```python
from build123d import *

# Parameters (mm, degrees)
BOSS_EXTRUDE1_DEPTH = 101.6
BOSS_EXTRUDE2_START = 50.8
BOSS_EXTRUDE2_DEPTH = 50.8
CUT_EXTRUDE1_DEPTH  = 800


with BuildPart() as part:
    # Sketch1 → Boss-Extrude1 (new body)
    with BuildSketch(Plane.XY):
        with BuildLine():
            Line((0, 254), (1473.2, 254))
            ThreePointArc((1473.2, 254), (1580.963073453, 209.363073453), (1625.6, 101.6))
            Line((1625.6, 101.6), (1625.6, -254))
            Line((1625.6, -254), (1623.6, -254))
            Line((1623.6, -254), (1623.6, 101.6))
            ThreePointArc((1623.6, 101.6), (1579.54885989, 207.94885989), (1473.2, 252))
            Line((1473.2, 252), (0, 252))
            ThreePointArc((0, 252), (-178.190908859, 178.190908859), (-252, 0))
            Line((-252, 0), (-254, 0))
            ThreePointArc((-254, 0), (-179.605122421, 179.605122421), (0, 254))
        make_face()
    extrude(amount=-BOSS_EXTRUDE1_DEPTH)

    # Sketch2 → Boss-Extrude2 (add)
    with BuildSketch(Plane.XY.offset(BOSS_EXTRUDE2_START)):
        with BuildLine():
            Line((1625.6, -254), (1625.6, 101.6))
            ThreePointArc((1625.6, 101.6), (1580.963073453, 209.363073453), (1473.2, 254))
            Line((1473.2, 254), (1320.8, 254))
            ThreePointArc((1320.8, 254), (1213.036926547, 209.363073453), (1168.4, 101.6))
            Line((1168.4, 101.6), (1168.4, -254))
            Line((1168.4, -254), (1170.4, -254))
            Line((1170.4, -254), (1170.4, 101.6))
            ThreePointArc((1170.4, 101.6), (1214.45114011, 207.94885989), (1320.8, 252))
            Line((1320.8, 252), (1473.2, 252))
            ThreePointArc((1473.2, 252), (1579.54885989, 207.94885989), (1623.6, 101.6))
            Line((1623.6, 101.6), (1623.6, -254))
            Line((1623.6, -254), (1625.6, -254))
        make_face()
    extrude(amount=-BOSS_EXTRUDE2_DEPTH)

    # Sketch3 → Cut-Extrude1 (cut)
    with BuildSketch(Plane(origin=(0, 0, 0), x_dir=(0, 0, -1), z_dir=(1, 0, 0))):
        with BuildLine():
            Line((101.6, 172.72), (101.6, 0))
            Line((101.6, 0), (0, 0))
            ThreePointArc((0, 0), (44.901280605, 18.598719395), (63.5, 63.5))
            Line((63.5, 63.5), (63.5, 134.62))
            ThreePointArc((63.5, 134.62), (74.659231637, 161.560768363), (101.6, 172.72))
        make_face()
    extrude(amount=-CUT_EXTRUDE1_DEPTH, mode=Mode.SUBTRACT)


solid = part.part
```
Design review of the part built by this model. Coordinates are the model's own, in mm. A direction names the side the tool comes from. Round coordinates to 2 decimals unless told otherwise and drop trailing zeros. Write each loop counter-clockwise with the first axis right and the second up, starting at its lowest first coordinate (ties: lowest second). Pieces come first, ordered by that corner, then holes. Notation, with made-up numbers: (85, 23.25) -> (140, 23.25) arc R31 cw to (140, 56.25) -> close; hole circle Ø5 at (19.5, 32). An arc over 180 degrees is marked (long way). Write item = value, one per line. Start each with the question number.
1) Take a section at C-C, the plane x = 1395. State the section outline as (y, z) points.
2) Take a section at B-B, the plane z = -41.5. State the section outline as (x, y) points.
3) Wall thickness on probe 1 along X at (y, z) = (58, 10); probe 2 along X at (y, z) = (-173, -31); probe 3 along Y at (x, z) = (896, -48): over which ranges is each line inside the solid? List them lowest first. Write a range as from..to.
4) Tool access review of faces 5 (the face through (-232, 99, -63.5)), 6 (the face through (1168.4, -74, 26)), 7 (the face through (1578.373, 209.112, -24.333)), 8 (the face through (-251.9, 18.4, -44.7)), 9 (the face through (1582.141, 208.172, -24.333)): name each direction out of +Z, -Z, +X, -X, +Y, -Y from which nothing blocks a thin tool from reaching the whole face with its end or side.
5) Take a section at A-A, the plane y = 197.5. State the section outline as (x, z) points.
6) Take a section at D-D, the plane y = 31.5. State the section outline as (x, z) points.
7) Mouldability with a two-part tool opening along X and no side actions: class faces 1 (the face through (1623.6, -74, -24)), 2 (the face through (-147.97, 206.45, -38.8)), 3 (the face through (1625.6, -79, -24)), 4 (the face through (747, 254, -41)) as +X half, -X half, draft (parallel to the pull), parting line (faces both ways), or undercut.
8) Clearance check with flat-ended pins moving along their axes: pin 1 (3 mm diameter, centred on x = 663, z = -18.5, fed in from -Y); pin 2 (2 mm diameter, centred on y = 187, z = -19, fed in from -X); pin 3 (16.5 mm diameter, centred on x = -231.5, y = 88.5, fed in from -Z). State where each tip first meets the part, or that it passes through.
Results list:
q1.outline = (252, -101.6) -> (254, -101.6) -> (254, 50.8) -> (252, 50.8) -> close
q2.outline = (-253.53, 15.44) -> (-251.53, 15.44) arc R252 cw to (0, 252) -> (1473.2, 252) arc R150.4 cw to (1623.6, 101.6) -> (1623.6, -254) -> (1625.6, -254) -> (1625.6, 101.6) arc R152.4 ccw to (1473.2, 254) -> (0, 254) arc R254 ccw to start
q3.probe_1 = 1168.4..1170.4, 1623.6..1625.6
q3.probe_2 = 1623.6..1625.6
q3.probe_3 = 252..254
q4.face_5 = -Z, -X, +Y, -Y
q4.face_6 = +Z, -Z, -X, +Y, -Y
q4.face_7 = +Z, -Z, -Y
q4.face_8 = -Z, -X, -Y
q4.face_9 = +Z, -Z, +X, +Y
q5.outline = (-159.72, -101.6) -> (-156.52, -101.6) -> (-156.52, 0) -> (-159.72, 0) -> close; (1202.36, 0) -> (1204.94, 0) -> (1204.94, 50.8) -> (1202.36, 50.8) -> close; (1589.06, -101.6) -> (1591.64, -101.6) -> (1591.64, 50.8) -> (1589.06, 50.8) -> close
q6.outline = (-252.04, -54.85) -> (-250.02, -54.85) -> (-250.02, 0) -> (-252.04, 0) -> close; (1168.4, 0) -> (1170.4, 0) -> (1170.4, 50.8) -> (1168.4, 50.8) -> close; (1623.6, -101.6) -> (1625.6, -101.6) -> (1625.6, 50.8) -> (1623.6, 50.8) -> close
q7.face_1 = undercut
q7.face_2 = -X half
q7.face_3 = +X half
q7.face_4 = draft
q8.pin_1 = 252
q8.pin_2 = -172.97
q8.pin_3 = -63.5
